Source: CAD feature listing. Evaluate the final solid. Frame: model axes, mm. A direction names the side the tool comes from. Round coordinates to 2 decimals unless told otherwise and drop trailing zeros. Loops run counter-clockwise (first coordinate to the right, second up) from the corner with the lowest first, then second, coordinate; pieces in that order, holes last. Notation, with made-up numbers: (34.25, 43) -> (82.25, 43) arc R19 cw to (82.25, 57) -> close; hole circle Ø4 at (25, 15.5). An arc over 180 degrees is marked (long way). Write item = value, one per line.
from build123d import *

# Parameters (mm, degrees)
SKETCH1_R           = 2
BOSS_EXTRUDE1_DEPTH = 10
SKETCH2_R           = 6.25
BOSS_EXTRUDE2_DEPTH = 24
SKETCH3_R           = 9
BOSS_EXTRUDE3_DEPTH = 10
CUT_EXTRUDE1_DEPTH  = 5


with BuildPart() as part:
    # Sketch1 → Boss-Extrude1 (new body)
    with BuildSketch(Plane(origin=(0, 0, 0), x_dir=(1, 0, 0), z_dir=(0, 1, 0))):
        with Locations(Location((0, 0, 0), (0, 0, 270))):
            Circle(SKETCH1_R)
    extrude(amount=BOSS_EXTRUDE1_DEPTH)

    # Sketch2 → Boss-Extrude2 (add)
    with BuildSketch(Plane(origin=(0, 10, 0), x_dir=(1, 0, 0), z_dir=(0, 1, 0))):
        with Locations(Location((0, 0, 0), (0, 0, 270))):
            Circle(SKETCH2_R)
    extrude(amount=BOSS_EXTRUDE2_DEPTH)

    # Sketch3 → Boss-Extrude3 (add)
    with BuildSketch(Plane(origin=(0, 34, 0), x_dir=(1, 0, 0), z_dir=(0, 1, 0))):
        with Locations(Location((0, 0, 0), (0, 0, 270))):
            Circle(SKETCH3_R)
    extrude(amount=BOSS_EXTRUDE3_DEPTH)

    # Sketch4 → Cut-Extrude1 (cut)
    with BuildSketch(Plane(origin=(0, 44, 0), x_dir=(1, 0, 0), z_dir=(0, 1, 0))):
        Polygon((0, 4.618802154), (-4, 2.309401077), (-4, -2.309401077), (0, -4.618802154), (4, -2.309401077), (4, 2.309401077), align=None)
    extrude(amount=-CUT_EXTRUDE1_DEPTH, mode=Mode.SUBTRACT)


solid = part.part
1. Section query B-B (y = 14). Return the cut outline in (x, z), then the cut area to 3 significant figures.
Evaluation:
outline = circle Ø12.5 at (0, 0)
area = 123 mm²
2. Set-up query: faces 4 (the face through (-2, 44, 4)), 5 (the face through (-1.87, 34, -6.13)), 6 (the face through (0, 39, 0)). Return all of +Z, -Z, +X, -X, +Y, -Y with unobstructed straight access to the full face (end or side cutting, diameter ignored); none if empty.
Evaluation:
face_4 = +Z, -Z, +X, -X, +Y
face_5 = -Y
face_6 = +Y
3. Contact query for flat-ended pins moving along their axis: pin 1 Ø4 at (x, y) = (4.5, 38) entering from +Z; pin 2 Ø5 at (y, z) = (18.5, 3.5) entering from +X; pin 3 Ø6.5 at (x, z) = (1.5, -0.5) entering from +Y; pin 4 Ø8 at (y, z) = (33, 7) entering from -X. Output: stop coordinate, or through.
Evaluation:
pin_1 = 8.65
pin_2 = 6.17
pin_3 = 44
pin_4 = -8.44
4. Section query A-A (z = 0). Return the cut outline in (x, y), then the cut area to 3 significant figures.
Evaluation:
outline = (-9, 34) -> (-6.25, 34) -> (-6.25, 10) -> (-2, 10) -> (-2, 0) -> (2, 0) -> (2, 10) -> (6.25, 10) -> (6.25, 34) -> (9, 34) -> (9, 44) -> (4, 44) -> (4, 39) -> (-4, 39) -> (-4, 44) -> (-9, 44) -> close
area = 480 mm²
5. Line query: probe 1 along Y at (x, z) = (-6.25, -5.5); probe 2 along Y at (x, z) = (2.5, -2.25); probe 3 along X at (y, z) = (40, -0.75). Output: solid intervals per line, ascending. Write a range as from..to.
Evaluation:
probe_1 = 34..44
probe_2 = 10..39
probe_3 = -8.97..-4, 4..8.97
6. Mould query, pull axis X, two halves, no side actions, for faces 1 (the face through (0, 0, 0)), 2 (the face through (-2, 5, 0)), 3 (the face through (1.97, 41.54, 3.48)). Classes: released by +X, released by -X, zero draft, split by the parting line, or undercut.
Evaluation:
face_1 = zero draft
face_2 = split by the parting line
face_3 = undercut
7. Section query D-D (z = 5.5). Return the cut outline in (x, y), then the cut area to 3 significant figures.
Evaluation:
outline = (-7.12, 34) -> (-2.97, 34) -> (-2.97, 10) -> (2.97, 10) -> (2.97, 34) -> (7.12, 34) -> (7.12, 44) -> (-7.12, 44) -> close
area = 285 mm²
8. Section query C-C (x = -1). Return the cut outline in (y, z), then the cut area to 3 significant figures.
Evaluation:
outline = (0, -1.73) -> (10, -1.73) -> (10, -6.17) -> (34, -6.17) -> (34, -8.94) -> (44, -8.94) -> (44, -4.04) -> (39, -4.04) -> (39, 4.04) -> (44, 4.04) -> (44, 8.94) -> (34, 8.94) -> (34, 6.17) -> (10, 6.17) -> (10, 1.73) -> (0, 1.73) -> close
area = 469 mm²
